from build123d import *

# Parameters (mm, degrees)
BOSS_EXTRUDE1_DEPTH = 20


with BuildPart() as part:
    # Sketch1 → Boss-Extrude1 (new body)
    with BuildSketch(Plane(origin=(0, 0, 0), x_dir=(1, 0, 0), z_dir=(0, 1, 0))):
        Polygon((-330, -655), (590, -655), (590, -415), (480, -415), (480, -10), (0, -10), (0, -415), (-330, -415), align=None)
    extrude(amount=BOSS_EXTRUDE1_DEPTH)


solid = part.part
Here's how the part is built. I have some questions about the finished solid (model axes, mm). A direction names the side the tool comes from. Round coordinates to 2 decimals unless told otherwise and drop trailing zeros. Loops run counter-clockwise (first coordinate to the right, second up) from the corner with the lowest first, then second, coordinate; pieces in that order, holes last.
1. We'd pull the mould along Z, two halves only. Please class faces 4 (the face through (-330, 10, 533)), 5 (the face through (536, 10, 415)), 6 (the face through (124, 10, 655)): +Z half, -Z half, draft (parallel to the pull), parting line (faces both ways), or undercut.
Answer list:
face 4: draft
face 5: -Z half
face 6: +Z half
2. If I drill on line 1 along Z through (x, y) = (497, 14.5); line 2 along X through (y, z) = (14.5, 41), over which ranges is the centre line in solid material (lowest first)?
Answer list:
line 1: z = 415 to 655
line 2: x = 0 to 480
3. Which directions (+Z, -Z, +X, -X, +Y, -Y) give clear straight access to the entire face, cutting with the end or side of a thin tool? Please do faces 1 (the face through (480, 10, 215)), 2 (the face through (243, 10, 10)), 3 (the face through (-163, 10, 415)).
Answer list:
face 1: -Z, +X, +Y, -Y
face 2: -Z, +X, -X, +Y, -Y
face 3: -Z, -X, +Y, -Y
4. If we section it at C-C on x = -130: Write out the boundary of the cut face in (y, z).
Answer list:
outline: (0, 415) - (20, 415) - (20, 655) - (0, 655) - close
5. For P1, Ø3, axis at y = 16.5, z = 197.5, coming from the -X side; P2, Ø10, axis at x = 553.5, y = 6, coming from the -Z side, each with a flat end and sliding along its axis, tell me the tip position at first contact or that it passes through.
Answer list:
P1: stops at x = 0
P2: stops at z = 415
6. If we section it at A-A on y = 4.75: Write out the boundary of the cut face in (x, z).
Answer list:
outline: (-330, 415) - (0, 415) - (0, 10) - (480, 10) - (480, 415) - (590, 415) - (590, 655) - (-330, 655) - close
7. If we section it at B-B on z = 210: Write out the boundary of the cut face in (x, y).
Answer list:
outline: (0, 0) - (480, 0) - (480, 20) - (0, 20) - close
